```python
from build123d import *

# Parameters (mm, degrees)
CUT_EXTRUDE1_DEPTH      = 18.391158693
CUT_EXTRUDE1_DEPTH_BACK = 18.391158693


with BuildPart() as part:
    # Sweep2: sweep along a path in Dimension Sketch
    with BuildLine(Plane.XY) as sweep2_path:
        Line((14.7, 1.15), (2.7, 1.15))
        ThreePointArc((2.7, 1.15), (2.133929691, 1.265530578), (1.658403483, 1.593642961))
        ThreePointArc((1.658403483, 1.593642961), (-2.3, 0), (1.658403483, -1.593642961))
        ThreePointArc((1.658403483, -1.593642961), (2.133929691, -1.265530578), (2.7, -1.15))
        Line((2.7, -1.15), (17.2, -1.15))
    # Sketch2 → Sweep2 (sweep)
    with BuildSketch(Plane(origin=(14.7, 1.15, 0), x_dir=(0, 0, 1), z_dir=(-1, 0, 0))):
        with BuildLine():
            Line((-1.149956521, -1.14), (1.149956521, -1.14))
            ThreePointArc((1.149956521, -1.14), (0, 0), (-1.149956521, -1.14))
        make_face()
    sweep(path=sweep2_path.line)

    # Sketch3 → Cut-Extrude1 (cut, two sides: drawn at the far end of the back side and taken through both)
    with BuildSketch(Plane.XY.offset(-CUT_EXTRUDE1_DEPTH_BACK)):
        Polygon((14.7, 0.57), (13.882315934, 1.15), (17.21, 1.15), (17.21, -1.15), (16.375313858, -1.15), (17.2, -0.58), (16.382315934, 0), (13.875313858, 0), align=None)
    extrude(amount=CUT_EXTRUDE1_DEPTH + CUT_EXTRUDE1_DEPTH_BACK, mode=Mode.SUBTRACT)


solid = part.part
```
Input: part model. Units: mm. Frame: model coordinates. A direction names the side the tool comes from. Give positions to 0.01 mm unless a question says otherwise; leave off trailing zeros. Write each loop counter-clockwise with the first axis right and the second up, starting at its lowest first coordinate (ties: lowest second). Pieces come first, ordered by that corner, then holes. Notation, with made-up numbers: (36.5, 87.25) - (60.5, 87.25) arc R17 cw to (60.5, 91.25) - close; hole circle Ø9 at (-29.5, 9). An arc over 180 degrees is marked (long way). Write item = value, one per line. Start each with the question number.
1) Pin query (flat end, axial travel): pin 1 (0.7 mm diameter, centred on x = 9.5, z = -0.5, fed in from -Y); pin 2 (1.5 mm diameter, centred on x = 2, y = 1, fed in from -Z). Return the tip coordinate at first contact, or that it passes through.
2) Draft query along Y for faces 1 (the face through (14.289, 0.286, -0.016)), 2 (the face through (10.05, -1.15, 0.03)), 3 (the face through (8.62, 1.15, 0.03)). Return one class per face: pulls with the +Y half, pulls with the -Y half, needs draft (parallel to the pull), parting line crosses it, or undercut.
3) Reachability of faces 4 (the face through (1.7, 0.21, 0.02)), 5 (the face through (16.87, -0.81, -0.01)) from +Z, -Z, +X, -X, +Y, -Y: full face, straight path, thin tool, end or side. Return the list, or none.
4) Material intervals for L1, parallel to Y at x = 0, z = 0.3; L2, parallel to Y at x = 0, z = 0.65; L3, parallel to X at y = 0.35, z = -0.15, sorted ascending. Write a range as [from, to].
5) Cut plane A-A (x = 13.5). Return loops of the section in (y, z), and give its area (3 significant figures).
Answers follow:
q1.pin_1 = -1.14
q1.pin_2 = -1.15
q2.face_1 = undercut
q2.face_2 = pulls with the -Y half
q2.face_3 = pulls with the +Y half
q3.face_4 = +Z, -Z
q3.face_5 = +Z, -Z, +X, -Y
q4.L1 = [-2.26, -1.16], [1.16, 2.26]
q4.L2 = [-2.1, -1.16], [1.16, 2.1]
q4.L3 = [-2.26, -1.11], [1.42, 14.38]
q5.outline = (-0.01, -1.15) - (-0.01, 1.15) arc R1.15 ccw to start; (0.01, -1.15) arc R1.15 ccw to (0.01, 1.15) - close
q5.area = 4.11 mm^2
